```python
from build123d import *

# Parameters (mm, degrees)
BASE_FLANGE_DEPTH      = 12
SPLIT_CLAMP_RING_DEPTH = 32
CLAMP_EAR_A_SKETCH_R   = 6
CLAMP_EAR_A_DEPTH      = 12
CLAMP_START            = -12
CLAMP_EAR_B_SKETCH_R   = 6
CLAMP_EAR_B_DEPTH      = 12


with BuildPart() as part:
    # Base Flange Sketch → Base Flange (new body)
    with BuildSketch(Plane(origin=(0, 0, 0), x_dir=(1, 0, 0), z_dir=(0, 1, 0))):
        with BuildLine():
            Line((-29.849623113, 3), (0, 3))
            Line((0, 3), (0, -3))
            Line((0, -3), (-29.849623113, -3))
            ThreePointArc((-29.849623113, -3), (-17.565731604, -24.319643772), (6.534455825, -29.279700939))
            Line((6.534455825, -29.279700939), (70.306891165, -15.047377923))
            ThreePointArc((70.306891165, -15.047377923), (73.681951889, -12.943680599), (75, -9.191437735))
            Line((75, -9.191437735), (75, -8))
            Line((75, -8), (50, -8))
            ThreePointArc((50, -8), (42, 0), (50, 8))
            Line((50, 8), (75, 8))
            Line((75, 8), (75, 9.191437735))
            ThreePointArc((75, 9.191437735), (73.681951889, 12.943680599), (70.306891165, 15.047377923))
            Line((70.306891165, 15.047377923), (6.534455825, 29.279700939))
            ThreePointArc((6.534455825, 29.279700939), (-17.565731604, 24.319643772), (-29.849623113, 3))
        make_face()
    extrude(amount=BASE_FLANGE_DEPTH)

    # Clamp Ring Sketch → Split Clamp Ring (add)
    with BuildSketch(Plane(origin=(0, 12, 0), x_dir=(1, 0, 0), z_dir=(0, 1, 0))):
        with BuildLine():
            ThreePointArc((6.534455825, 29.279700939), (-17.565731604, 24.319643772), (-29.849623113, 3))
            Line((-29.849623113, 3), (-18.761663039, 3))
            ThreePointArc((-18.761663039, 3), (19, 0), (-18.761663039, -3))
            Line((-18.761663039, -3), (-29.849623113, -3))
            ThreePointArc((-29.849623113, -3), (-17.565731604, -24.319643772), (6.534455825, -29.279700939))
            ThreePointArc((6.534455825, -29.279700939), (30, 0), (6.534455825, 29.279700939))
        make_face()
    extrude(amount=SPLIT_CLAMP_RING_DEPTH)

    # Clamp Ear A Sketch → Clamp Ear A (add)
    with BuildSketch(Plane.XY.offset(3)):
        with BuildLine():
            Line((-36, 36), (-25, 36))
            Line((-25, 36), (-25, 8))
            Line((-25, 8), (-36, 8))
            ThreePointArc((-36, 8), (-50, 22), (-36, 36))
        make_face()
        with Locations((-36, 22)):
            Circle(CLAMP_EAR_A_SKETCH_R, mode=Mode.SUBTRACT)
    extrude(amount=CLAMP_EAR_A_DEPTH)

    # Clamp Ear B Sketch → Clamp Ear B (add)
    with BuildSketch(Plane.XY.offset(-3).offset(CLAMP_START)):
        with BuildLine():
            Line((-36, 36), (-25, 36))
            Line((-25, 36), (-25, 8))
            Line((-25, 8), (-36, 8))
            ThreePointArc((-36, 8), (-50, 22), (-36, 36))
        make_face()
        with Locations((-36, 22)):
            Circle(CLAMP_EAR_B_SKETCH_R, mode=Mode.SUBTRACT)
    extrude(amount=CLAMP_EAR_B_DEPTH)


solid = part.part
```
For this review, take the finished solid that the model builds, in its own axes (mm). A direction names the side the tool comes from. Round coordinates to 2 decimals unless told otherwise and drop trailing zeros. Loops run counter-clockwise (first coordinate to the right, second up) from the corner with the lowest first, then second, coordinate; pieces in that order, holes last.
Q1. Mouldability with a two-part tool opening along Z and no side actions: class faces 6 (the face through (18.983, 27.776, -0.793)), 7 (the face through (41, 12, 0)), 8 (the face through (38.867, 5.916, -22.064)) as +Z half, -Z half, draft (parallel to the pull), parting line (faces both ways), or undercut.
Result sheet:
face 6: undercut
face 7: draft
face 8: -Z half
Q2. To check wall thickness, follow line 1 along Y through (x, z) = (-36, -6.5); line 2 along Z through (x, y) = (0, 32); line 3 along Z through (x, y) = (-28.5, 27). State the ranges of each line that lie inside material, in increasing order.
Result sheet:
line 1: y = 8 to 16, 28 to 36
line 2: z = -30 to -19, 19 to 30
line 3: z = -15 to -3, 3 to 15
Q3. Add section A-A on y = 22. Write out the cut boundary in (x, z).
Result sheet:
outline: (-50, -15) - (-42, -15) - (-42, -3) - (-50, -3) - close; (-50, 3) - (-42, 3) - (-42, 15) - (-50, 15) - close; (-30, -15) - (-25.98, -15) arc R30 ccw (long way) to (-25.98, 15) - (-30, 15) - (-30, 3) - (-18.76, 3) arc R19 cw (long way) to (-18.76, -3) - (-30, -3) - close
Q4. Machinability: for faces 1 (the face through (4, 12, 0)), 2 (the face through (-38, 16, -15)), 3 (the face through (-32, 36, -9)), 4 (the face through (-25, 17, -3)), 5 (the face through (62, 6, -8)), which of the approach directions +Z, -Z, +X, -X, +Y, -Y give a long, thin tool a straight path to every point of the face, cutting with its end or side? Answer none if there is none.
Result sheet:
face 1: +Y
face 2: -Z, -X, +Y, -Y
face 3: -Z, -X, +Y
face 4: -X, +Y, -Y
face 5: +X, +Y, -Y
Q5. Add section B-B on x = 46.5. Write out the cut boundary in (y, z).
Result sheet:
outline: (0, -20.36) - (12, -20.36) - (12, -7.19) - (0, -7.19) - close; (0, 7.19) - (12, 7.19) - (12, 20.36) - (0, 20.36) - close
Q6. Insertion check: pin 1 Ø11 at (x, y) = (-36, 22) entering from -Z; pin 2 Ø12 at (x, y) = (-42, 22) entering from -Z; pin 3 Ø7 at (x, y) = (-42.5, 20.5) entering from +Z; pin 4 Ø8 at (x, y) = (-1, 15) entering from -Z. Each pin has a flat end and moves straight along its axis. Give the tip position at first contact, or say it passes through.
Result sheet:
pin 1: passes through
pin 2: stops at z = -15
pin 3: stops at z = 15
pin 4: stops at z = -30
Q7. Add section D-D on x = -38. Write out the cut boundary in (y, z), plus the area to 3 significant figures.
Result sheet:
outline: (8.14, -15) - (16.34, -15) - (16.34, -3) - (8.14, -3) - close; (8.14, 3) - (16.34, 3) - (16.34, 15) - (8.14, 15) - close; (27.66, -15) - (35.86, -15) - (35.86, -3) - (27.66, -3) - close; (27.66, 3) - (35.86, 3) - (35.86, 15) - (27.66, 15) - close
area: 394 mm2
Q8. Add section C-C on y = 5.5. Write out the cut boundary in (x, z), plus the area to 3 significant figures.
Result sheet:
outline: (-29.85, -3) arc R30 ccw to (6.53, -29.28) - (70.31, -15.05) arc R6 ccw to (75, -9.19) - (75, -8) - (50, -8) arc R8 cw to (50, 8) - (75, 8) - (75, 9.19) arc R6 ccw to (70.31, 15.05) - (6.53, 29.28) arc R30 ccw to (-29.85, 3) - (0, 3) - (0, -3) - close
area: 4,080 mm2
